For this review, use the dimensioned drawing (mm, ordinates from the lowest corner) and the shaded views. A direction names the side the tool comes from. Give positions to 0.01 mm unless a question says otherwise; leave off trailing zeros. Write each loop counter-clockwise with the first axis right and the second up, starting at its lowest first coordinate (ties: lowest second). Pieces come first, ordered by that corner, then holes. Notation, with made-up numbers: M -7.75,16.5 L 23.25,16.5 A34 ccw 23.25,53.5 Z; hole C 69.5,-14 d3. An arc over 180 degrees is marked long. Write each question's results on one line, items separated by ' | '. Start each with the question number.
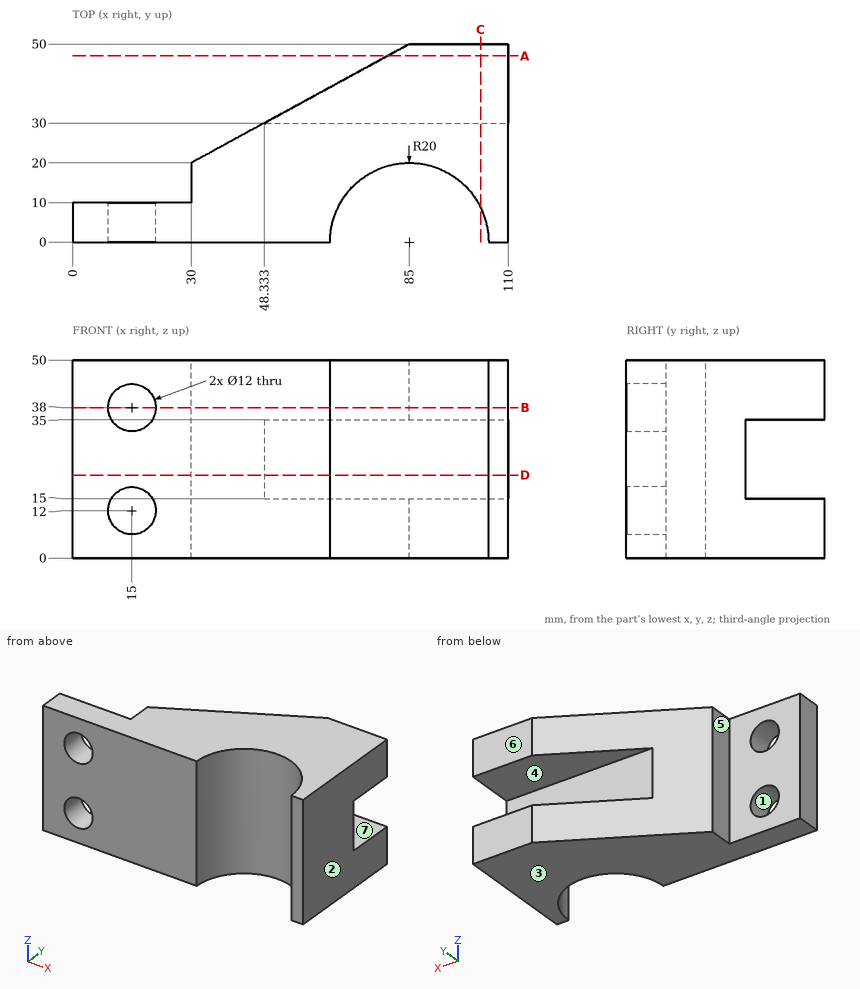
(1) Add section D-D (z = 21). State the section outline as (x, y) points, then the cut area to 3 significant figures.
(2) Add section C-C (x = 103). State the section outline as (y, z) points, then the cut area to 3 significant figures.
(3) Add section A-A (y = 47). State the section outline as (x, z) points, then the cut area to 3 significant figures.
(4) Machinability: for the marked faces 5, 6 and 7, which of the approach directions +Z, -Z, +X, -X, +Y, -Y give a long, thin tool a straight path to every point of the face, cutting with its end or side? Answer none if there is none.
(5) Draft analysis for pull direction Z (two halves, no side actions). For the marked faces 1, 2, 3 and 4, state which applies: pulls with the +Z half, pulls with the -Z half, needs draft (parallel to the pull), parting line crosses it, or undercut.
(6) Clearance check with flat-ended pins moving along their axes: P1, Ø11, axis at x = 15, z = 12, coming from the -Y side; P2, Ø5, axis at y = 17.5, z = 24.5, coming from the -X side; P3, Ø4, axis at y = 36, z = 34, coming from the +X side; P4, Ø3, axis at x = 55.5, z = 8, coming from the +Y side. State where each tip first meets the part, or that it passes through.
(7) Add section B-B (z = 38). State the section outline as (x, y) points.
(8) Wall thickness on L1, parallel to X at y = 2, z = 38; L2, parallel to X at y = 4, z = 38 (1 decimal); L3, parallel to Y at x = 56, z = 16.5: over which ranges is each line inside the solid? List them lowest first.
Calculated:
1) outline: M 0,0 L 65,0 A20 cw 105,0 L 110,0 L 110,30 L 48.33,30 L 30,20 L 30,10 L 0,10 Z | area: 1,980 mm²
2) outline: M 8.72,0 L 50,0 L 50,15 L 30,15 L 30,35 L 50,35 L 50,50 L 8.72,50 Z | area: 1,660 mm²
3) outline: M 79.5,0 L 110,0 L 110,15 L 79.5,15 Z; M 79.5,35 L 110,35 L 110,50 L 79.5,50 Z | area: 915 mm²
4) face 5: +Z, -Z, -X, +Y | face 6: +Z, -Z, +X, -X, +Y | face 7: +X, -X, +Y
5) face 1: undercut | face 2: needs draft | face 3: pulls with the -Z half | face 4: undercut
6) P1: passes through | P2: stops at x = 30 | P3: stops at x = 110 | P4: stops at y = 34.73
7) outline: M 0,0 L 9,0 L 9,10 L 0,10 Z; M 21,0 L 65,0 A20 cw 105,0 L 110,0 L 110,50 L 85,50 L 30,20 L 30,10 L 21,10 Z
8) L1: x = 0 to 9, 21 to 65.1, 104.9 to 110 | L2: x = 0 to 9, 21 to 65.4, 104.6 to 110 | L3: y = 0 to 30
